For this review, take the finished solid that the model builds, in its own axes (mm). Face numbers are marked on the shaded views. Round coordinates to 2 decimals unless told otherwise and drop trailing zeros. Loops run counter-clockwise (first coordinate to the right, second up) from the corner with the lowest first, then second, coordinate; pieces in that order, holes last.
1) Insertion check: pin 1 (1.5 mm diameter, centred on x = -36.5, z = -38, fed in from -Y); pin 2 (1 mm diameter, centred on x = 4, z = -16, fed in from +Y); pin 3 (6 mm diameter, centred on x = 66.5, y = 157, fed in from +Z). Each pin has a flat end and moves straight along its axis. Give the tip position at first contact, or say it passes through.
2) Take a section at C-C (y = 117). Give the number of separate pieces and of enclosed holes in the cut face, then the cut area to 3 significant figures.
3) Take a section at D-D (z = 0). State the section outline as (x, y) points.
4) Take a section at B-B (x = 3). State the section outline as (y, z) points (3 decimals).
5) Take a section at A-A (y = 0). State the section outline as (x, z) points.
6) Mouldability with a two-part tool opening along Y and no side actions: class the marked faces 1, 2 and 3 as pulls with the +Y half, pulls with the -Y half, needs draft (parallel to the pull), parting line crosses it, or undercut.
7) Wall thickness on L1, parallel to X at y = 5.5, z = -6; L2, parallel to Z at x = -74, y = 117; L3, parallel to Y at x = -68.5, z = -128.5: over which ranges is each line inside the solid? List them lowest first.
```python
from build123d import *

# Parameters (mm, degrees)
SKETCH1_R           = 25
BOSS_EXTRUDE1_DEPTH = 7.5
BOSS_EXTRUDE2_DEPTH = 7.5
BOSS_EXTRUDE4_DEPTH = 12
FILLET1_R           = 20


with BuildPart() as part:
    # Sketch1 → Boss-Extrude1 (new, symmetric)
    with BuildSketch(Plane(origin=(0, 0, 0), x_dir=(0, 0, -1), z_dir=(1, 0, 0))):
        Circle(SKETCH1_R)
    extrude(amount=BOSS_EXTRUDE1_DEPTH, both=True)

    # Sketch2 → Boss-Extrude2 (add, symmetric)
    with BuildSketch(Plane(origin=(0, 0, 0), x_dir=(0, 0, -1), z_dir=(1, 0, 0))):
        Polygon((-25, 0), (-11.852856042, 35.333850942), (33.197452276, 162.153435325), (42.115400597, 158.580697497), (39.917408227, 141.125260536), (3.66577496, -1.999651309), align=None)
    extrude(amount=BOSS_EXTRUDE2_DEPTH, both=True)

    # Sketch4 → Boss-Extrude4 (add)
    with BuildSketch(Plane(origin=(0, 151.187639508, -60.569290091), x_dir=(1, 0, 0), z_dir=(0, 0.9282770434137098, -0.3718894065056191))):
        with BuildLine():
            Line((67.852060571, 102.029312181), (67.852060571, 49.967186724))
            ThreePointArc((67.852060571, 49.967186724), (0, -17.884873847), (-67.852060571, 49.967186724))
            Line((-67.852060571, 49.967186724), (-67.852060571, 102.029312181))
            ThreePointArc((-67.852060571, 102.029312181), (-73.482108128, 109.670210388), (-82.447891925, 106.556453525))
            ThreePointArc((-82.447891925, 106.556453525), (0, -50.032813276), (82.447891925, 106.556453525))
            ThreePointArc((82.447891925, 106.556453525), (73.482108128, 109.670210388), (67.852060571, 102.029312181))
        make_face()
    extrude(amount=BOSS_EXTRUDE4_DEPTH)

    # Fillet1
    fillet1_edges = [part.edges().sort_by_distance(p)[0] for p in [
        (0, 162.153435325, -33.197452276),
    ]]
    fillet(fillet1_edges, radius=FILLET1_R)


solid = part.part
```
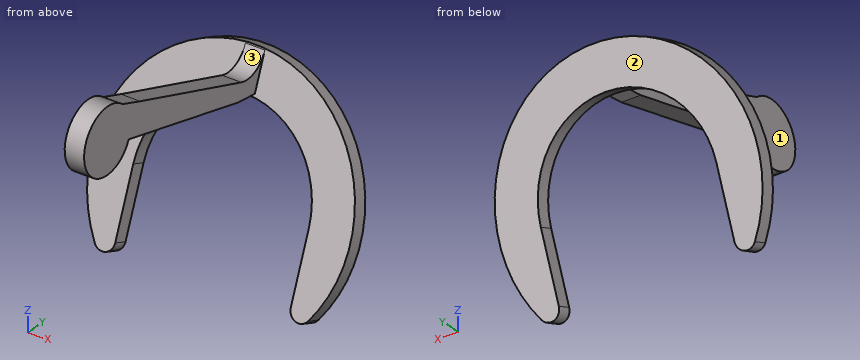
Response:
1. pin 1: stops at y = 159.93
1. pin 2: stops at y = 175.51
1. pin 3: stops at z = -38.57
2. separate pieces: 3
2. enclosed holes: 0
2. area: 914 mm2
3. outline: (-7.5, -25) - (7.5, -25) - (7.5, 68.7) - (-7.5, 68.7) - close
4. outline: (16.342, 18.92) arc R25 ccw (long way) to (22.922, -9.978) - (141.125, -39.917) - (158.581, -42.115) - (157.814, -44.029) - (168.953, -48.491) - (180.917, -18.629) - (169.778, -14.167) - (169.302, -15.355) arc R20 cw to (144.041, -26.763) - (35.334, 11.853) - close
5. outline: (-7.5, -25) - (7.5, -25) - (7.5, 25) - (-7.5, 25) - close
6. face 1: needs draft
6. face 2: pulls with the +Y half
6. face 3: undercut
7. L1: x = -7.5 to 7.5
7. L2: z = -165.17 to -145.91
7. L3: y = 123.97 to 136.9
